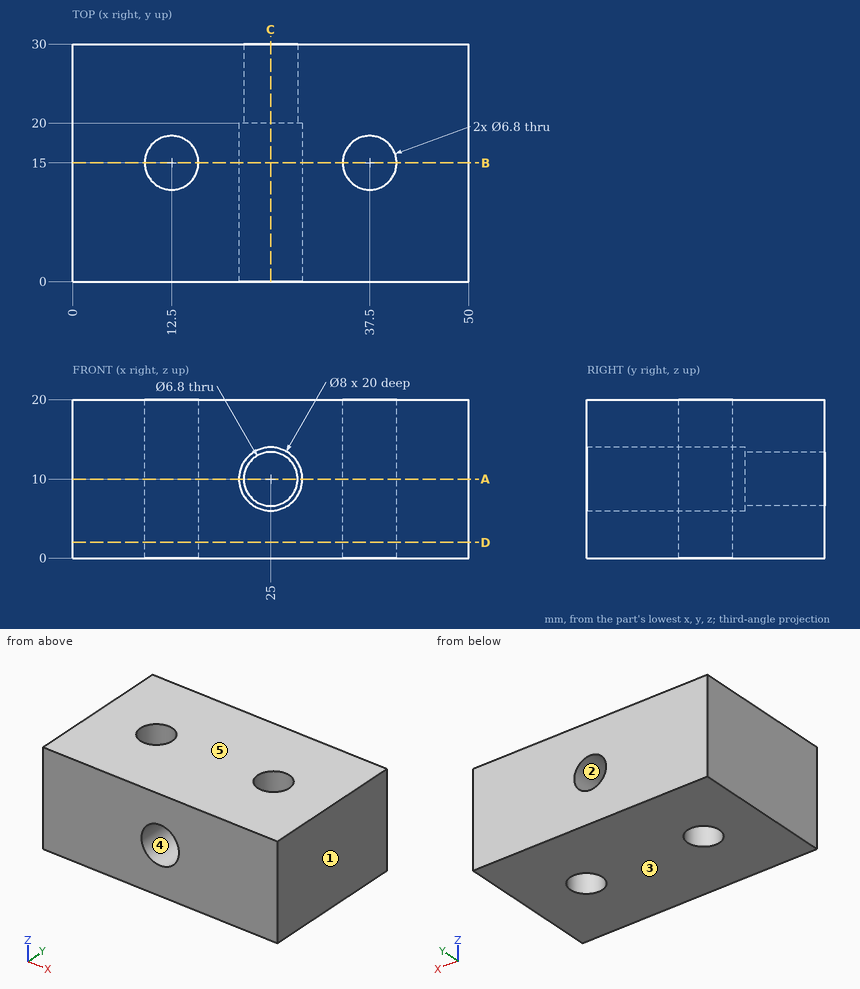
Print and shaded views of the part. All mm, measured from the part's lowest x, y and z. A direction names the side the tool comes from. Coordinates: 2 decimals unless noted, no trailing zeros. Loops run counter-clockwise (first coordinate to the right, second up) from the corner with the lowest first, then second, coordinate; pieces in that order, holes last. Notation, with made-up numbers: (24.25, 86) -> (73.25, 86) arc R26 cw to (73.25, 109) -> close; hole circle Ø10 at (-24, -7). An arc over 180 degrees is marked (long way). Use a Markdown table: item, result. Add a question column.
Item 1: Probe probe 1 along Y at (x, z) = (12.5, 10.25); probe 2 along X at (y, z) = (24.5, 10); probe 3 along X at (y, z) = (16, 16.5). List the from-to ranges inside material, lowest first.
Item 2: Pull direction Z, two halves, no side cores. Call the marked faces 1, 2 and 3: +Z half, -Z half, draft (parallel to the pull), parting line (faces both ways), or undercut.
Item 3: Flat gauge pin, fed straight in: P1, Ø4, axis at x = 12.5, y = 15, coming from the +Z side. Where does the tip first touch, or does it go through?
Item 4: Band-saw the part on A-A on z = 10. Write the cut outline in (x, y), plus the area to 3 significant figures.
Item 5: Which spindle directions (+Z, -Z, +X, -X, +Y, -Y) get a long thin tool onto all of the face, cutting with end or side? Do the marked faces 4 and 5. Say none if no direction does.
Item 6: Band-saw the part on B-B on y = 15. Write the cut outline in (x, z).
Item 7: Band-saw the part on D-D on z = 2. Write the cut outline in (x, y).
Item 8: Band-saw the part on C-C on x = 25. Write the cut outline in (y, z), plus the area to 3 significant figures.
Geometry says:
| question | item | result |
|---|---|---|
| 1 | probe 1 | 0 to 11.6, 18.4 to 30 |
| 1 | probe 2 | 0 to 21.6, 28.4 to 50 |
| 1 | probe 3 | 0 to 9.25, 15.75 to 34.25, 40.75 to 50 |
| 2 | face 1 | draft |
| 2 | face 2 | undercut |
| 2 | face 3 | -Z half |
| 3 | P1 | through |
| 4 | outline | (0, 0) -> (21, 0) -> (21, 20) -> (21.6, 20) -> (21.6, 30) -> (0, 30) -> close; (28.4, 20) -> (29, 20) -> (29, 0) -> (50, 0) -> (50, 30) -> (28.4, 30) -> close; hole circle Ø6.8 at (12.5, 15); hole circle Ø6.8 at (37.5, 15) |
| 4 | area | 1,200 mm² |
| 5 | face 4 | -Y |
| 5 | face 5 | +Z, +X, -X, +Y, -Y |
| 6 | outline | (0, 0) -> (9.1, 0) -> (9.1, 20) -> (0, 20) -> close; (15.9, 0) -> (34.1, 0) -> (34.1, 20) -> (15.9, 20) -> close; (40.9, 0) -> (50, 0) -> (50, 20) -> (40.9, 20) -> close; hole circle Ø8 at (25, 10) |
| 7 | outline | (0, 0) -> (50, 0) -> (50, 30) -> (0, 30) -> close; hole circle Ø6.8 at (12.5, 15); hole circle Ø6.8 at (37.5, 15) |
| 8 | outline | (0, 0) -> (30, 0) -> (30, 6.6) -> (20, 6.6) -> (20, 6) -> (0, 6) -> close; (0, 14) -> (20, 14) -> (20, 13.4) -> (30, 13.4) -> (30, 20) -> (0, 20) -> close |
| 8 | area | 372 mm² |
